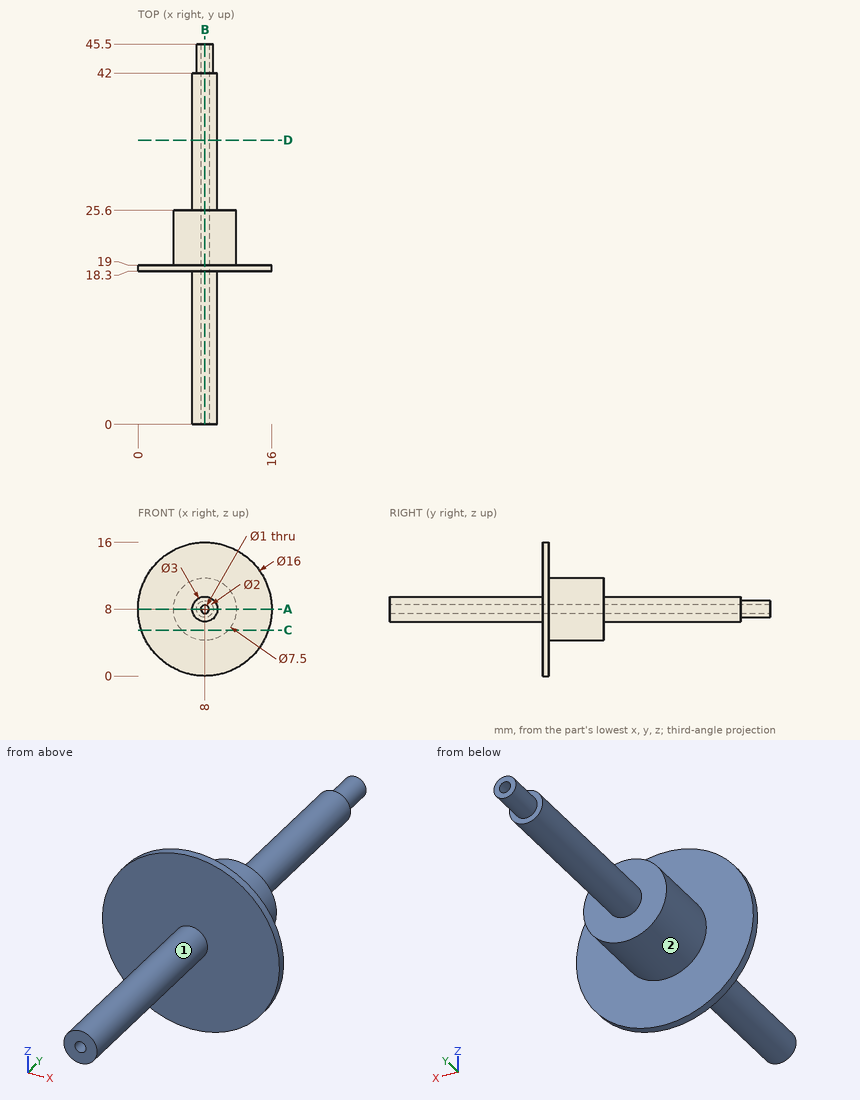
Answer from the drawing. Dimensions are ordinates in mm from the lowest x, y and z of the part. A direction names the side the tool comes from. Give positions to 0.01 mm unless a question says otherwise; leave off trailing zeros. Order: outer loops, then holes, each group sorted by start corner. A loop starts at its lowest first (then second) coordinate and runs counter-clockwise, first axis right, second up.
(1) Find section B-B (x = 8). Give the vertices of the cut face in (y, z).
(2) Find section D-D (y = 34). Give the vertices of the cut face in (x, z), plus the area to 3 significant figures.
(3) Given pin 1 (1.5 mm diameter, centred on y = 18, z = 7, fed in from -X); pin 2 (5 mm diameter, centred on x = 11, y = 30.5, fed in from -Z); pin 3 (6 mm diameter, centred on x = 2, z = 6.5, fed in from +Y), each flat-ended and moving along its own axis, determine where each tip first touches the part or whether it passes through.
(4) Find section A-A (z = 8). Give the vertices of the cut face in (x, y).
(5) Straight lines are drawn through the part: L1, parallel to X at y = 20.5, z = 8; L2, parallel to Y at x = 14.5, z = 11.5; L3, parallel to X at y = 34.5, z = 8. For each, find the intervals that lie inside material, in ascending order.
(6) Find section C-C (z = 5.5). Give the vertices of the cut face in (x, y), plus the area to 3 significant figures.
(7) For the marked faces 1 and 2, determine the directions among +Z, -Z, +X, -X, +Y, -Y from which every point of the face is accessible in a straight line to the end or side of a thin tool.
Result sheet:
1. outline: (0, 6.5) - (18.3, 6.5) - (18.3, 0) - (19, 0) - (19, 4.25) - (25.6, 4.25) - (25.6, 6.5) - (42, 6.5) - (42, 7) - (45.5, 7) - (45.5, 7.5) - (0, 7.5) - close; (0, 8.5) - (45.5, 8.5) - (45.5, 9) - (42, 9) - (42, 9.5) - (25.6, 9.5) - (25.6, 11.75) - (19, 11.75) - (19, 16) - (18.3, 16) - (18.3, 9.5) - (0, 9.5) - close
2. outline: circle Ø3 at (8, 8); hole circle Ø1 at (8, 8)
2. area: 6.28 mm2
3. pin 1: stops at x = 0.01
3. pin 2: stops at z = 6.59
3. pin 3: stops at y = 25.6
4. outline: (0, 18.3) - (6.5, 18.3) - (6.5, 0) - (7.5, 0) - (7.5, 45.5) - (7, 45.5) - (7, 42) - (6.5, 42) - (6.5, 25.6) - (4.25, 25.6) - (4.25, 19) - (0, 19) - close; (8.5, 0) - (9.5, 0) - (9.5, 18.3) - (16, 18.3) - (16, 19) - (11.75, 19) - (11.75, 25.6) - (9.5, 25.6) - (9.5, 42) - (9, 42) - (9, 45.5) - (8.5, 45.5) - close
5. L1: x = 4.25 to 7.5, 8.5 to 11.75
5. L2: y = 18.3 to 19
5. L3: x = 6.5 to 7.5, 8.5 to 9.5
6. outline: (0.4, 18.3) - (15.6, 18.3) - (15.6, 19) - (10.8, 19) - (10.8, 25.6) - (5.2, 25.6) - (5.2, 19) - (0.4, 19) - close
6. area: 47.5 mm2
7. face 1: -Y
7. face 2: +Y
